from build123d import *

# Parameters (mm, degrees)
SKETCH1_W            = 406
SKETCH1_H            = 372
BOSS_EXTRUDE1_DEPTH  = 5
SKETCH2_W            = 282.5
SKETCH2_H            = 83
CUT_EXTRUDE1_DEPTH   = 276.372475022
M5_CLEARANCE_HOLE1_D = 5.5
FILLET1_SIZE         = 2


with BuildPart() as part:
    # Sketch1 → Boss-Extrude1 (new body)
    with BuildSketch(Plane.XY):
        Rectangle(SKETCH1_W, SKETCH1_H)
    extrude(amount=BOSS_EXTRUDE1_DEPTH)

    # Sketch2 → Cut-Extrude1 (cut, through all)
    with BuildSketch(Plane.XY.offset(5)):
        with Locations((33.75, -144.5)):
            Rectangle(SKETCH2_W, SKETCH2_H)
    extrude(amount=-CUT_EXTRUDE1_DEPTH, mode=Mode.SUBTRACT)

    # M5 Clearance Hole1 (through all)
    with Locations(Plane.XY.offset(5)):
        with Locations((-17.5, -30), (17.5, -30)):
            Hole(M5_CLEARANCE_HOLE1_D / 2)

    # Fillet1
    fillet1_edges = [part.edges().sort_by_distance(p)[0] for p in [
        (-107.5, -186, 2.5),
        (-107.5, -103, 2.5),
        (175, -103, 2.5),
        (175, -186, 2.5),
        (-203, 186, 2.5),
        (203, 186, 2.5),
        (203, -186, 2.5),
        (-203, -186, 2.5),
    ]]
    chamfer(fillet1_edges, length=FILLET1_SIZE)


solid = part.part
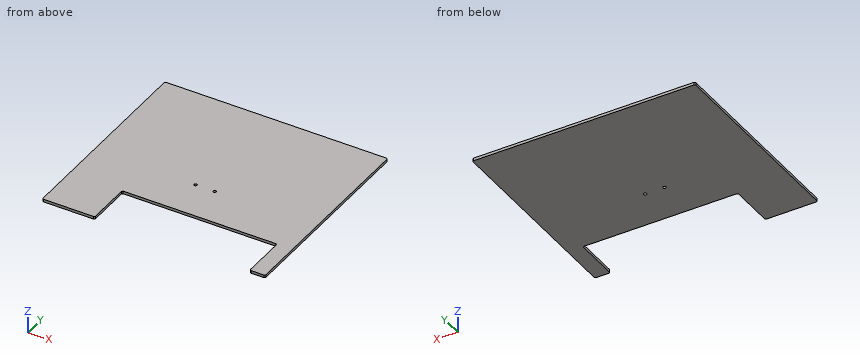
Model file for the job. Use its own axes, mm. Coordinates: 2 decimals unless noted, no trailing zeros. Order: outer loops, then holes, each group sorted by start corner. A loop starts at its lowest first (then second) coordinate and runs counter-clockwise, first axis right, second up. Notation, with made-up numbers: (12, 62.5) -> (62, 62.5) arc R20 cw to (62, 88.5) -> close; hole circle Ø7 at (55, 9.25). An arc over 180 degrees is marked (long way). Return JSON: item names as keys, results as strings. Group by question number.
Item 1: Wall check: line 1 along X through (y, z) = (-139, 2.95); line 2 along Y through (x, z) = (17.5, 1.8); line 3 along Y through (x, z) = (132, 4.75). Give the ranges that are in metal, low to high. Write a range as [from, to].
Item 2: Saw through at B-B on y = -128. Write the cut outline in (x, z), then the cut area to 4 significant figures.
Item 3: Flat gauge pins, fed straight in: P1, Ø1.5, axis at x = -8, z = 3, coming from the -Y side; P2, Ø3.5, axis at x = -17.5, y = -30, coming from the +Z side. Where does each tip first touch, or does it go through?
Item 4: Saw through at C-C on x = -85. Write the cut outline in (y, z).
Item 5: Saw through at A-A on z = 1.75. Write the cut outline in (x, y).
Values found:
{
 "1": {"line 1": "x = [-203, -107.5], [175, 203]", "line 2": "y = [-103, -32.75], [-27.25, 186]", "line 3": "y = [-103, 186]"},
 "2": {"outline": "(-203, 0) -> (-107.5, 0) -> (-107.5, 5) -> (-203, 5) -> close; (175, 0) -> (203, 0) -> (203, 5) -> (175, 5) -> close", "area": "617.5 mm2"},
 "3": {"P1": "stops at y = -103", "P2": "passes through"},
 "4": {"outline": "(-103, 0) -> (186, 0) -> (186, 5) -> (-103, 5) -> close"},
 "5": {"outline": "(-203, -184) -> (-201, -186) -> (-109.5, -186) -> (-107.5, -184) -> (-107.5, -105) -> (-105.5, -103) -> (173, -103) -> (175, -105) -> (175, -184) -> (177, -186) -> (201, -186) -> (203, -184) -> (203, 184) -> (201, 186) -> (-201, 186) -> (-203, 184) -> close; hole circle Ø5.5 at (-17.5, -30); hole circle Ø5.5 at (17.5, -30)"}
}
